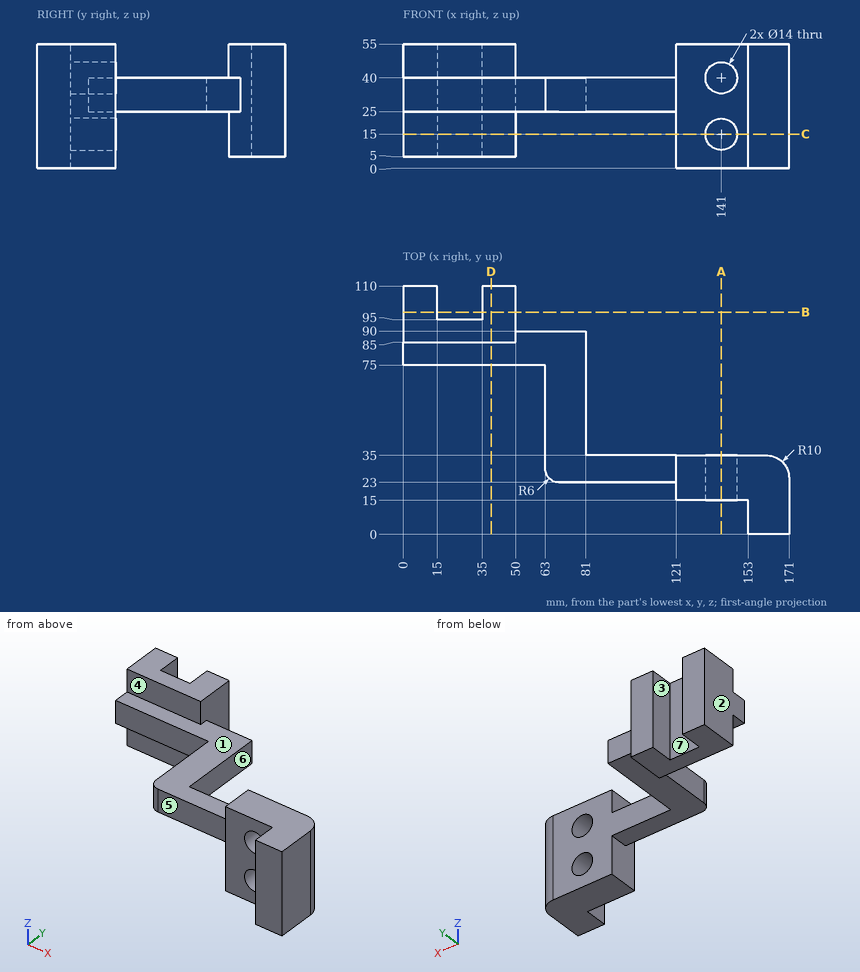
Here's the drawing with two shaded views (mm, measured from the low corner). I have some questions. A direction names the side the tool comes from. Round coordinates to 2 decimals unless told otherwise and drop trailing zeros. Order: outer loops, then holes, each group sorted by start corner. A loop starts at its lowest first (then second) coordinate and runs counter-clockwise, first axis right, second up. Notation, with made-up numbers: M -35.75,-14 L 3.25,-14 A31 ccw 3.25,22 Z; hole C -14,35 d7. An arc over 180 degrees is marked long. Answer in a Markdown table with one row per item.
Item 1: Imagine slicing it at B-B, the plane y = 98.5. Write out the boundary of the cut face in (x, z), and give its area (3 significant figures).
A:
| item | result |
|---|---|
| outline | M 0,5 L 15,5 L 15,55 L 0,55 Z; M 35,5 L 50,5 L 50,55 L 35,55 Z |
| area | 1,500 mm2 |
Item 2: Thinking about a two-plate mould opening in X: for the marked faces 1, 2 and 3, which applies, +X half, -X half, draft (parallel to the pull), parting line (faces both ways), or undercut?
A:
| item | result |
|---|---|
| face 1 | draft |
| face 2 | -X half |
| face 3 | undercut |
Item 3: Imagine slicing it at D-D, the plane x = 39. Write out the boundary of the cut face in (y, z).
A:
| item | result |
|---|---|
| outline | M 75,25 L 85,25 L 85,5 L 110,5 L 110,55 L 85,55 L 85,40 L 75,40 Z |
Item 4: Imagine slicing it at A-A, the plane x = 141. Write out the boundary of the cut face in (y, z), and give its area (3 significant figures).
A:
| item | result |
|---|---|
| outline | M 15,0 L 35,0 L 35,8 L 15,8 Z; M 15,22 L 35,22 L 35,33 L 15,33 Z; M 15,47 L 35,47 L 35,55 L 15,55 Z |
| area | 540 mm2 |
Item 5: If I drill on L1, parallel to Y at x = 125, z = 49; L2, parallel to X at y = 5, z = 46; L3, parallel to X at y = 29, z = 15, over which ranges is the centre line in solid material (lowest first)? Write a range as from..to.
A:
| item | result |
|---|---|
| L1 | y = 15..35 |
| L2 | x = 153..171 |
| L3 | x = 121..134, 148..170.17 |
Item 6: Imagine slicing it at C-C, the plane z = 15. Write out the boundary of the cut face in (x, y), and give its area (3 significant figures).
A:
| item | result |
|---|---|
| outline | M 0,85 L 50,85 L 50,110 L 35,110 L 35,95 L 15,95 L 15,110 L 0,110 Z; M 121,15 L 134,15 L 134,35 L 121,35 Z; M 148,15 L 153,15 L 153,0 L 171,0 L 171,25 A10 ccw 161,35 L 148,35 Z |
| area | 1,920 mm2 |
Item 7: For the marked faces 4, 5, 6 and 7, which set-ups out of +Z, -Z, +X, -X, +Y, -Y let a thin tool reach every point of the face, with its end or its side?
A:
| item | result |
|---|---|
| face 4 | +Z, +X, -X, -Y |
| face 5 | +Z, -Z, -X, -Y |
| face 6 | +Z, -Z, +X, +Y |
| face 7 | +Z, -Z, +Y |
Item 8: I'm going to push flat-ended pins straight in: pin 1 (3 mm diameter, centred on y = 83.5, z = 32, fed in from +X); pin 2 (12.5 mm diameter, centred on y = 102, z = 22.5, fed in from +X); pin 3 (12 mm diameter, centred on x = 72, z = 34, fed in from +Y); pin 4 (7.5 mm diameter, centred on y = 100.5, z = 22, fed in from -X). Where does each tip first touch, or does it pass through?
A:
| item | result |
|---|---|
| pin 1 | stops at x = 81 |
| pin 2 | stops at x = 50 |
| pin 3 | stops at y = 90 |
| pin 4 | stops at x = 0 |
